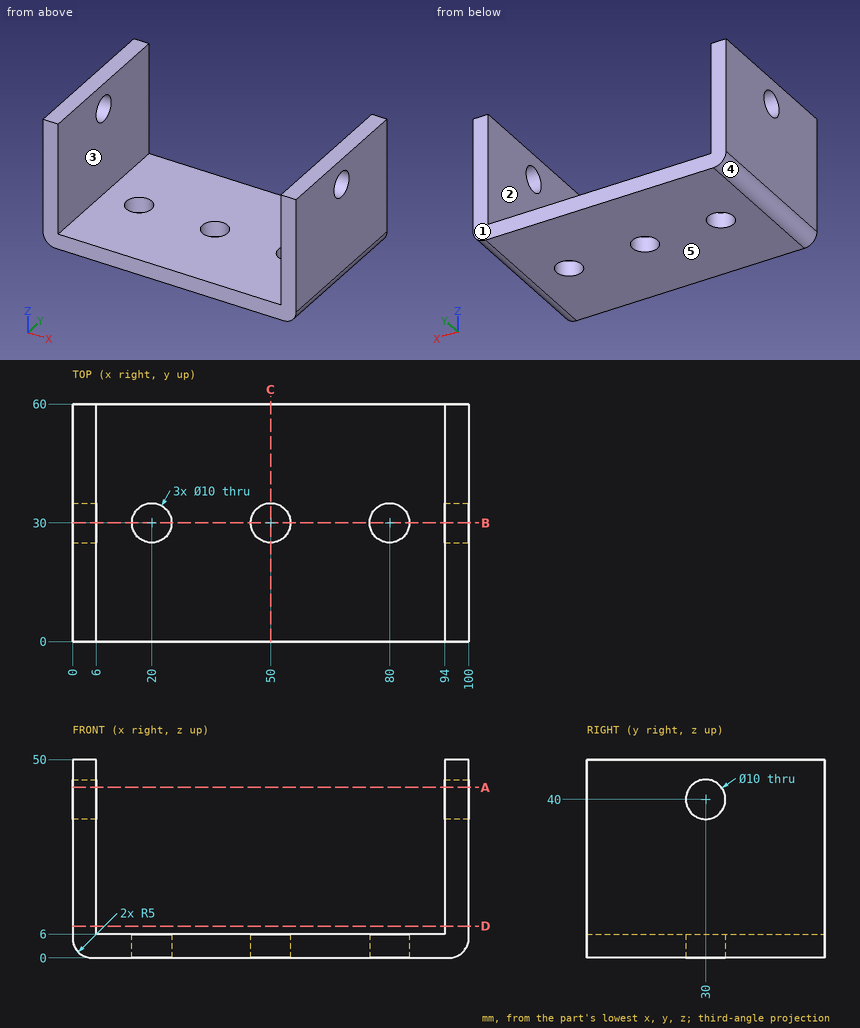
Answer from the drawing. Dimensions are ordinates in mm from the lowest x, y and z of the part. A direction names the side the tool comes from. Round coordinates to 2 decimals unless told otherwise and drop trailing zeros. Order: outer loops, then holes, each group sorted by start corner. A loop starts at its lowest first (then second) coordinate and runs counter-clockwise, first axis right, second up. Notation, with made-up numbers: (-7.5, -8.75) - (30.5, -8.75) arc R22 ccw to (30.5, 29.25) - close; hole circle Ø7 at (33.5, 61). An arc over 180 degrees is marked (long way). Put each result on its own line as item: value. Start each with the question number.
(1) Find section D-D (z = 8). Give the vertices of the cut face in (x, y).
(2) For the marked faces 1 and 2, determine the directions among +Z, -Z, +X, -X, +Y, -Y from which every point of the face is accessible in a straight line to the end or side of a thin tool.
(3) Find section A-A (z = 43). Give the vertices of the cut face in (x, y), plus the area to 3 significant figures.
(4) Find section B-B (y = 30). State how many separate pieces and enclosed holes the cut face has, plus the area to 3 significant figures.
(5) Find section C-C (x = 50). Give the vertices of the cut face in (y, z).
(6) Given P1, Ø3, axis at x = 86, y = 32.5, coming from the -Z side; P2, Ø13, axis at x = 50, y = 30, coming from the +Z side, each flat-ended and moving along its own axis, determine where each tip first touches the part or whether it passes through.
(7) Straight lines are drawn through the part: probe 1 along Y at (x, z) = (80, 3); probe 2 along X at (y, z) = (46, 47); probe 3 along Z at (x, y) = (9, 10). For each, find the intervals that lie inside material, in ascending order. Write a range as from..to.
(8) Determine the mould class of the marked faces 3, 4 and 5 for opening direction X: released by +X, released by -X, zero draft, split by the parting line, or undercut.
Reply:
1. outline: (0, 0) - (6, 0) - (6, 60) - (0, 60) - close; (94, 0) - (100, 0) - (100, 60) - (94, 60) - close
2. face 1: +Z, -Z, +X, -X, +Y
2. face 2: +Z, +Y, -Y
3. outline: (0, 0) - (6, 0) - (6, 26) - (0, 26) - close; (0, 34) - (6, 34) - (6, 60) - (0, 60) - close; (94, 0) - (100, 0) - (100, 26) - (94, 26) - close; (94, 34) - (100, 34) - (100, 60) - (94, 60) - close
3. area: 624 mm^2
4. separate pieces: 6
4. enclosed holes: 0
4. area: 817 mm^2
5. outline: (0, 0) - (25, 0) - (25, 6) - (0, 6) - close; (35, 0) - (60, 0) - (60, 6) - (35, 6) - close
6. P1: z = 0
6. P2: z = 6
7. probe 1: 0..25, 35..60
7. probe 2: 0..6, 94..100
7. probe 3: 0..6
8. face 3: undercut
8. face 4: released by -X
8. face 5: zero draft
